Design review of the part built by this model. Coordinates are the model's own, in mm. Give positions to 0.01 mm unless a question says otherwise; leave off trailing zeros. Loops run counter-clockwise (first coordinate to the right, second up) from the corner with the lowest first, then second, coordinate; pieces in that order, holes last. Notation, with made-up numbers: (38.5, 46) -> (82.5, 46) arc R32 ccw to (82.5, 76) -> close; hole circle Ø2 at (-9, 73.5). An arc over 180 degrees is marked (long way). Use CSV: the item, a comma, the result in double quotes. Start each with the question number.
Item 1: We need section D-D (y = -27.5). State the section outline as (x, z) points.
Item 2: We need section C-C (z = 2.3). State the section outline as (x, y) points.
Item 3: We need section B-B (y = 0). State the section outline as (x, z) points, plus the area to 3 significant figures.
Item 4: We need section A-A (x = 0). State the section outline as (y, z) points, plus the area to 3 significant figures.
Item 5: Wall thickness on line 1 along X through (y, z) = (-50, 4.45); line 2 along X through (y, z) = (-48.5, 1.65); line 3 along X through (y, z) = (-39.5, 1.2): over which ranges is each line inside the solid? List them lowest first. Write a range as from..to.
Item 6: Clearance check with flat-ended pins moving along their axes: pin 1 (1 mm diameter, centred on y = -2.5, z = 2.5, fed in from -X); pin 2 (1 mm diameter, centred on y = -36.5, z = 2.5, fed in from -X); pin 3 (1.5 mm diameter, centred on x = -4.5, z = 2.5, fed in from +Y). State where each tip first meets the part, or that it passes through.
from build123d import *

# Parameters (mm, degrees)
SKETCH1_R           = 2.6
BOSS_EXTRUDE1_DEPTH = 5


with BuildPart() as part:
    # Sketch1 → Boss-Extrude1 (new body)
    with BuildSketch(Plane.XY):
        with BuildLine():
            Line((42.024169285, -45.949384393), (6.103781177, 4.358194046))
            ThreePointArc((6.103781177, 4.358194046), (1.532383005, 7.341784683), (-3.850823854, 6.435926945))
            Line((-3.850823854, 6.435926945), (-87.930468078, -43.871651494))
            ThreePointArc((-87.930468078, -43.871651494), (-91.308733105, -52.305145448), (-84.079644224, -57.807578439))
            Line((-84.079644224, -57.807578439), (-24.079629528, -57.807578439))
            Line((-24.079629528, -57.807578439), (35.920388108, -57.807578439))
            ThreePointArc((35.920388108, -57.807578439), (42.588838278, -53.740037081), (42.024169285, -45.949384393))
        make_face()
        with Locations((-84.079644224, -50.307578439)):
            Circle(SKETCH1_R, mode=Mode.SUBTRACT)
        with Locations((-24.079629528, -50.307578439)):
            Circle(SKETCH1_R, mode=Mode.SUBTRACT)
        with Locations((35.920388108, -50.307578439)):
            Circle(SKETCH1_R, mode=Mode.SUBTRACT)
        Circle(SKETCH1_R, mode=Mode.SUBTRACT)
        with BuildLine():
            Line((-5.346611856, -9.025717813), (-50.457391397, -36.016960475))
            ThreePointArc((-50.457391397, -36.016960475), (-52.709568082, -41.639289778), (-47.890175494, -45.307578439))
            Line((-47.890175494, -45.307578439), (-24.079629528, -45.307578439))
            Line((-24.079629528, -45.307578439), (16.492768241, -45.307578439))
            ThreePointArc((16.492768241, -45.307578439), (20.938401688, -42.5958842), (20.561955693, -37.402115742))
            Line((20.561955693, -37.402115742), (1.289791498, -10.41087308))
            ThreePointArc((1.289791498, -10.41087308), (-1.757807283, -8.421812655), (-5.346611856, -9.025717813))
        make_face(mode=Mode.SUBTRACT)
    extrude(amount=BOSS_EXTRUDE1_DEPTH)


solid = part.part
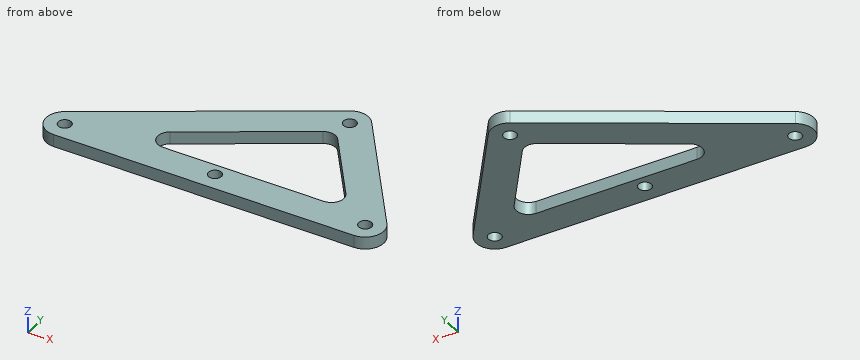
Results found:
1,outline,"(-60.57, 0) -> (-36.22, 0) -> (-36.22, 5) -> (-60.57, 5) -> close; (13.49, 0) -> (28.85, 0) -> (28.85, 5) -> (13.49, 5) -> close"
2,outline,"(-87.93, -43.87) arc R7.5 ccw to (-84.08, -57.81) -> (35.92, -57.81) arc R7.5 ccw to (42.02, -45.95) -> (6.1, 4.36) arc R7.5 ccw to (-3.85, 6.44) -> close; hole circle Ø5.2 at (-84.08, -50.31); hole (-50.46, -36.02) arc R5 ccw to (-47.89, -45.31) -> (16.49, -45.31) arc R5 ccw to (20.56, -37.4) -> (1.29, -10.41) arc R5 ccw to (-5.35, -9.03) -> close; hole circle Ø5.2 at (-24.08, -50.31); hole circle Ø5.2 at (0, 0); hole circle Ø5.2 at (35.92, -50.31)"
3,outline,"(-14.61, 0) -> (-2.6, 0) -> (-2.6, 5) -> (-14.61, 5) -> close; (2.6, 0) -> (9.22, 0) -> (9.22, 5) -> (2.6, 5) -> close"
3,area,"93.1 mm²"
4,outline,"(-57.81, 0) -> (-45.31, 0) -> (-45.31, 5) -> (-57.81, 5) -> close; (-9.16, 0) -> (-2.6, 0) -> (-2.6, 5) -> (-9.16, 5) -> close; (2.6, 0) -> (7.5, 0) -> (7.5, 5) -> (2.6, 5) -> close"
4,area,"120 mm²"
5,line 1,"-91.57..-86.66, -81.5..-26.66, -21.5..33.34, 38.5..43.41"
5,line 2,"-91.36..-85.95, -82.21..-25.95, -22.21..34.05, 37.79..43.2"
5,line 3,"-80.62..-52.82, 21.43..37.42"
6,pin 1,"x = -19.62"
6,pin 2,"x = -76.45"
6,pin 3,"y = 6.5"
